```python
from build123d import *

# Parameters (mm, degrees)
FILLET1_R = 0.6
FILLET2_R = 0.6


with BuildPart() as part:
    # Sketch1 → Revolve1 (revolve)
    with BuildSketch(Plane.XY, mode=Mode.PRIVATE) as revolve1_sk:
        Polygon((0, 17.5), (10, 17.5), (10, 20.2), (9.565, 20.2), (9.565, 24.9), (10, 24.9), (10, 27.5), (0, 27.5), (0, 24.9), (0.435, 24.9), (0.435, 20.2), (0, 20.2), align=None)
    revolve(revolve1_sk.sketch.rotate(Axis((0, 0, 0), (1, 0, 0)), 90), axis=Axis((0, 0, 0), (1, 0, 0)))

    # Fillet1
    fillet1_edges = [part.edges().sort_by_distance(p)[0] for p in [
        (0, 0, -27.5),
        (10, 0, -27.5),
    ]]
    fillet(fillet1_edges, radius=FILLET1_R)

    # Fillet2
    fillet2_edges = [part.edges().sort_by_distance(p)[0] for p in [
        (10, 0, -17.5),
        (0, 0, -17.5),
    ]]
    fillet(fillet2_edges, radius=FILLET2_R)


solid = part.part
```
Can you work these out from the model? Positions are in its coordinate system, mm. A direction names the side the tool comes from. Round coordinates to 2 decimals unless told otherwise and drop trailing zeros. Loops run counter-clockwise (first coordinate to the right, second up) from the corner with the lowest first, then second, coordinate; pieces in that order, holes last. Notation, with made-up numbers: M 61.25,-23.5 L 109.25,-23.5 A28 cw 109.25,2.5 Z; hole C 79.25,79 d1. An arc over 180 degrees is marked long. Write item = value, one per line. Start each with the question number.
(1) Suppose I cut it at C-C on x = 7.5. Write out the boundary of the cut face in (y, z), plus the area to 3 significant figures.
(2) If we mould it in two halves opening along Z, with no side actions, what happens to faces 1 (the face through (0, -8, -17)), 2 (the face through (0.21, 17.92, 9.32)), 3 (the face through (9.78, 17.92, 9.32)), 4 (the face through (4.938, 24.397, 12.69))? For each: released by +Z, released by -Z, zero draft, split by the parting line, or undercut.
(3) I need wall thicknesses on line 1 along Y through (x, z) = (0.15, 0); line 2 along Y through (x, z) = (4.75, 0); line 3 along X through (y, z) = (-17, 14.5) (3 decimals). Which ranges of each line are inside material? Lowest first, please.
(4) I'm going to push flat-ended pins straight in: P1, Ø12, axis at y = 19.5, z = 8.5, coming from the -X side; P2, Ø2, axis at x = 4, y = -14.5, coming from the +Z side; P3, Ø2, axis at x = 3, y = 17.5, coming from the -Z side; P4, Ø5, axis at x = 2, z = -17, coming from the +Y side. Where does each tip first touch, or does it pass through?
(5) Which directions (+Z, -Z, +X, -X, +Y, -Y) give clear straight access to the entire face, cutting with the end or side of a thin tool? Please do faces 5 (the face through (9.79, 15.15, -19.76)), 6 (the face through (5.062, 17.084, -3.794)), 7 (the face through (0.435, -20.4, -0.1)).
Answer block:
q1.outline = C 0,0 d55; hole C 0,0 d35
q1.area = 1,410 mm²
q2.face_1 = zero draft
q2.face_2 = undercut
q2.face_3 = undercut
q2.face_4 = split by the parting line
q3.line_1 = -27.3 to -24.9, -20.2 to -17.7, 17.7 to 20.2, 24.9 to 27.3
q3.line_2 = -27.5 to -17.5, 17.5 to 27.5
q3.line_3 = 0.435 to 9.565
q4.P1 = 0
q4.P2 = 23.96
q4.P3 = -22
q4.P4 = 23.37
q5.face_5 = +X
q5.face_6 = +X, -X
q5.face_7 = -X
